from build123d import *

# Parameters (mm, degrees)
SKETCH_1_R      = 20
EXTRUDE_1_DEPTH = 15
SKETCH_3_W      = 3
SKETCH_3_H      = 8
EXTRUDE_3_DEPTH = 15
CHAMFER_2_SIZE  = 0.5


with BuildPart() as part:
    # 草图1 → 凸台-拉伸1 (new body)
    with BuildSketch(Plane(origin=(0, 0, 0), x_dir=(1, 0, 0), z_dir=(0, 1, 0))):
        with BuildLine():
            Line((-135, 30), (-135, -30))
            Line((-135, -30), (0, -30))
            ThreePointArc((0, -30), (30, 0), (0, 30))
            Line((0, 30), (-135, 30))
        make_face()
        with Locations(Location((0, 0, 0), (0, 0, 270))):
            Circle(SKETCH_1_R, mode=Mode.SUBTRACT)
        with BuildLine():
            Line((-124.75, 5.25), (-119.75, 5.25))
            ThreePointArc((-119.75, 5.25), (-114.5, 0), (-119.75, -5.25))
            Line((-119.75, -5.25), (-124.75, -5.25))
            ThreePointArc((-124.75, -5.25), (-130, 0), (-124.75, 5.25))
        make_face(mode=Mode.SUBTRACT)
        with BuildLine():
            Line((-99.75, 5.25), (-94.75, 5.25))
            ThreePointArc((-94.75, 5.25), (-89.5, 0), (-94.75, -5.25))
            Line((-94.75, -5.25), (-99.75, -5.25))
            ThreePointArc((-99.75, -5.25), (-105, 0), (-99.75, 5.25))
        make_face(mode=Mode.SUBTRACT)
    extrude(amount=EXTRUDE_1_DEPTH)

    # 草图3 → 凸台-拉伸3 (add, through all)
    with BuildSketch(Plane.XZ):
        with Locations((-136.5, 26)):
            Rectangle(SKETCH_3_W, SKETCH_3_H)
    extrude(amount=-EXTRUDE_3_DEPTH)

    # 倒角2
    chamfer_2_edges = [part.edges().sort_by_distance(p)[0] for p in [
        (-67.5, 15, -30),
        (0, 0, -20),
        (0, 15, -20),
        (-135, 15, -4),
        (-130, 0, 0),
        (-122.25, 0, 5.25),
        (-114.5, 0, 0),
        (-122.25, 0, -5.25),
        (-130, 15, 0),
        (-122.25, 15, 5.25),
        (-114.5, 15, 0),
        (-122.25, 15, -5.25),
        (-105, 0, 0),
        (-97.25, 0, 5.25),
        (-89.5, 0, 0),
        (-97.25, 0, -5.25),
        (-105, 15, 0),
        (-97.25, 15, 5.25),
        (-89.5, 15, 0),
        (-97.25, 15, -5.25),
        (-69, 15, 30),
        (-135, 0, -4),
        (-136.5, 15, 22),
        (-138, 15, 26),
        (-138, 7.5, 22),
        (-138, 7.5, 30),
        (-67.5, 0, -30),
        (-138, 0, 26),
        (-136.5, 0, 22),
        (30, 0, 0),
        (-69, 0, 30),
        (30, 15, 0),
        (-135, 7.5, -30),
    ]]
    chamfer(chamfer_2_edges, length=CHAMFER_2_SIZE)


solid = part.part
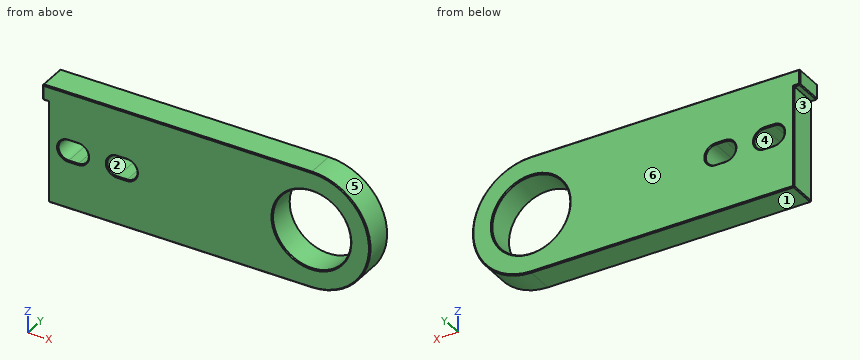
Input: part model. Units: mm. Frame: model coordinates. Face numbers are marked on the shaded views. A direction names the side the tool comes from. Give positions to 0.01 mm unless a question says otherwise; leave off trailing zeros. Order: outer loops, then holes, each group sorted by start corner. A loop starts at its lowest first (then second) coordinate and runs counter-clockwise, first axis right, second up. Notation, with made-up numbers: (-14.75, -1) -> (36.25, -1) arc R22 cw to (36.25, 11) -> close; hole circle Ø11 at (55.5, -40). An arc over 180 degrees is marked (long way). Use one line per item in the form item = value.
1) Section A-A, the plane z = 0. Count the separate pieces of the cut face and the enclosed holes in it, and give its area (3 significant figures).
Response values:
separate_pieces = 4
enclosed_holes = 0
area = 1,410 mm^2
2) Section B-B, the plane y = 7. Return loops of the section in (x, z), and give its area (3 significant figures).
Response values:
outline = (-138, 22.5) -> (-137.5, 22) -> (-135, 22) -> (-135, -29.5) -> (-134.5, -30) -> (0, -30) arc R30 ccw to (0, 30) -> (-137.5, 30) -> (-138, 29.5) -> close; hole (-124.75, -5.25) -> (-119.75, -5.25) arc R5.25 ccw to (-119.75, 5.25) -> (-124.75, 5.25) arc R5.25 ccw to start; hole (-99.75, -5.25) -> (-94.75, -5.25) arc R5.25 ccw to (-94.75, 5.25) -> (-99.75, 5.25) arc R5.25 ccw to start; hole circle Ø40 at (0, 0)
area = 8,000 mm^2
3) First-contact query: pin 1 Ø1.5 at (y, z) = (5, -2.5) entering from -X; pin 2 Ø1.2 at (x, y) = (-136.5, 6) entering from -Z. Flat tips, straight axial feed; report the tip coordinate or a pass-through.
Response values:
pin_1 = -135
pin_2 = 22
4) Reachability of the marked faces 1 and 2 from +Z, -Z, +X, -X, +Y, -Y: full face, straight path, thin tool, end or side. Return the list, or none.
Response values:
face_1 = -Z, +X, -X, +Y, -Y
face_2 = +Y, -Y
5) Line query: probe 1 along X at (y, z) = (5, 0); probe 2 along Z at (x, y) = (9.5, 9.75); probe 3 along X at (y, z) = (7.5, -1.5). Output: solid intervals per line, ascending.
Response values:
probe_1 = -135 to -130, -114.5 to -105, -89.5 to -20, 20 to 30
probe_2 = -28.46 to -17.6, 17.6 to 28.46
probe_3 = -135 to -129.78, -114.72 to -104.78, -89.72 to -19.94, 19.94 to 29.96
6) Mould query, pull axis X, two halves, no side actions, for the marked faces 3, 4, 5 and 6. Classes: pulls with the +X half, pulls with the -X half, needs draft (parallel to the pull), parting line crosses it, or undercut.
Response values:
face_3 = pulls with the -X half
face_4 = undercut
face_5 = pulls with the +X half
face_6 = needs draft
